Work out the finished part from the listing and answer in its coordinate system (mm). Round coordinates to 2 decimals unless told otherwise and drop trailing zeros. Loops run counter-clockwise (first coordinate to the right, second up) from the corner with the lowest first, then second, coordinate; pieces in that order, holes last. Notation, with made-up numbers: (39.25, -30.75) - (65.25, -30.75) arc R24 cw to (65.25, 0.25) - close; hole circle Ø5 at (-33.75, 7.25). An arc over 180 degrees is marked (long way). Use CSV: the item, a comma, the result in double quotes. Start each with the question number.
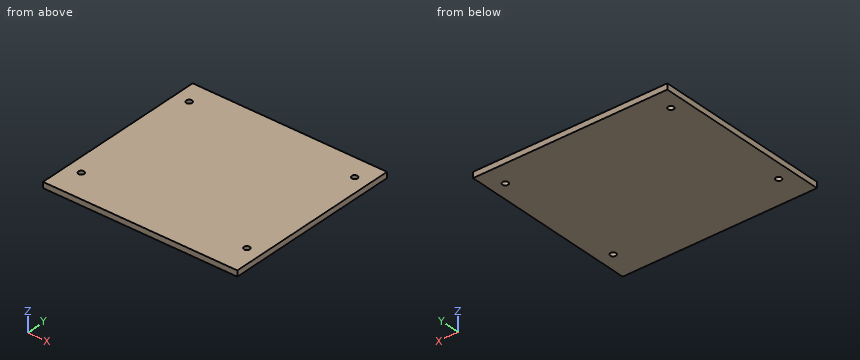
from build123d import *

# Parameters (mm, degrees)
SKETCH_1_W          = 270
SKETCH_1_H          = 250
EXTRUDE_1_DEPTH     = 8
SKETCH_2_R          = 4
CUT_EXTRUDE_1_DEPTH = 10


with BuildPart() as part:
    # 草图1 → 凸台-拉伸1 (new body)
    with BuildSketch(Plane.XY):
        with Locations((135, -125)):
            Rectangle(SKETCH_1_W, SKETCH_1_H)
    extrude(amount=EXTRUDE_1_DEPTH)

    # 草图2 → 切除-拉伸1 (cut)
    with BuildSketch(Plane.XY.offset(8)):
        with Locations((250, -30)):
            Circle(SKETCH_2_R)
        with Locations((250, -210)):
            Circle(SKETCH_2_R)
        with Locations((20, -210)):
            Circle(SKETCH_2_R)
        with Locations((20, -30)):
            Circle(SKETCH_2_R)
    extrude(amount=-CUT_EXTRUDE_1_DEPTH, mode=Mode.SUBTRACT)


solid = part.part
Item 1: A cutting plane is placed at A-A (y = -210). Determine the outline of the cut face in (x, z).
Item 2: A cutting plane is placed at B-B (x = 250). Determine the outline of the cut face in (y, z), plus the area to 3 significant figures.
Item 3: Find the intervals of material crossed by probe 1 along Y at (x, z) = (250, 6.25); probe 2 along X at (y, z) = (-26.5, 1); probe 3 along X at (y, z) = (-209, 6), in increasing order. Write a range as [from, to].
Item 4: This flat-tipped pin is pushed along its axis until it touches: pin 1 Ø5 at (x, y) = (20, -30) entering from +Z. Where does it stop, or does it pass through?
Result sheet:
1,outline,"(0, 0) - (16, 0) - (16, 8) - (0, 8) - close; (24, 0) - (246, 0) - (246, 8) - (24, 8) - close; (254, 0) - (270, 0) - (270, 8) - (254, 8) - close"
2,outline,"(-250, 0) - (-214, 0) - (-214, 8) - (-250, 8) - close; (-206, 0) - (-34, 0) - (-34, 8) - (-206, 8) - close; (-26, 0) - (0, 0) - (0, 8) - (-26, 8) - close"
2,area,"1,870 mm^2"
3,probe 1,"[-250, -214], [-206, -34], [-26, 0]"
3,probe 2,"[0, 18.06], [21.94, 248.06], [251.94, 270]"
3,probe 3,"[0, 16.13], [23.87, 246.13], [253.87, 270]"
4,pin 1,"through"
